Here's how the part is built. I have some questions about the finished solid (model axes, mm). Give positions to 0.01 mm unless a question says otherwise; leave off trailing zeros. Order: outer loops, then holes, each group sorted by start corner. A loop starts at its lowest first (then second) coordinate and runs counter-clockwise, first axis right, second up. Notation, with made-up numbers: (54, 0.5) - (62, 0.5) arc R23 cw to (62, 13.5) - close; hole circle Ø11 at (-16, 9.25). An arc over 180 degrees is marked (long way). One line per question, with ' | ' between items.
from build123d import *

# Parameters (mm, degrees)
SWEEP1_PROFILE_R   = 3
CUT_EXTRUDE1_DEPTH = 25


with BuildPart() as part:
    # Sweep1: sweep along a path in Sketch1
    with BuildLine(Plane.XY) as sweep1_path:
        ThreePointArc((-91.040352938, 214.477630854), (-194.295396542, 128.601317578), (-233, 0))
    # Sweep1 profile (on start of the path) → Sweep1 (sweep)
    with BuildSketch(Plane(origin=(-91.040352938, 214.477630854, 0), x_dir=(0.39073112848927155, -0.9205048534524413, 0), z_dir=(-0.9205048534524413, -0.39073112848927155, 0))):
        Circle(SWEEP1_PROFILE_R)
    sweep(path=sweep1_path.line)

    # Sketch6 → Cut-Extrude1 (cut, symmetric)
    with BuildSketch(Plane.XY):
        with BuildLine():
            Line((0, 0), (-230.569138435, 14.102212633))
            ThreePointArc((-230.569138435, 14.102212633), (-230.892259483, 7.054396551), (-231, 0))
            Line((-231, 0), (0, 0))
        make_face()
        with BuildLine():
            Line((0, 0), (-90.258890681, 212.636621148))
            ThreePointArc((-90.258890681, 212.636621148), (-138.212982732, 185.089630732), (-178.245278763, 146.934068884))
            Line((-178.245278763, 146.934068884), (0, 0))
        make_face()
    extrude(amount=CUT_EXTRUDE1_DEPTH, both=True, mode=Mode.SUBTRACT)


solid = part.part
1) Please list where these lines run through material, in increasing order: L1, parallel to Z at x = -222, y = 69.5; L2, parallel to X at y = 10.5, z = 0.5; L3, parallel to Y at x = -130.5, z = 1.5.
Model answer:
L1: z = -2.98 to 2.98 | L2: x = -235.72 to -230.76 | L3: y = 190.61 to 196.15
2) I want a section at A-A (z = 1.25). List the corners of the cut face in (x, y) for me, plus the area to 3 significant figures.
Model answer:
outline: (-235.73, 0) - (-231, 0) arc R231 cw to (-230.57, 14.1) - (-229.84, 14.06) arc R230.27 cw to (-177.68, 146.47) - (-178.25, 146.93) arc R231 cw to (-90.26, 212.64) - (-92.11, 216.99) arc R235.73 ccw to start | area: 1,400 mm2
3) I'm going to push flat-ended pins straight in: P1, Ø12, axis at x = -144.5, y = 173.5, coming from the -Z side; P2, Ø1, axis at y = 102.5, z = 0.5, coming from the -X side; P3, Ø1.5, axis at x = -184, z = 0.5, coming from the +Y side. Where does each tip first touch, or does it pass through?
Model answer:
P1: stops at z = -2.75 | P2: stops at x = -212.79 | P3: stops at y = 148.66
